Study the drawing (mm; zero at the part's minimum x, y, z) and answer. Coordinates: 2 decimals unless noted, no trailing zeros. Loops run counter-clockwise (first coordinate to the right, second up) from the corner with the lowest first, then second, coordinate; pieces in that order, holes last. Notation, with made-up numbers: M 28.25,76 L 49.25,76 A24 ccw 49.25,106 Z; hole C 52,31.25 d1. An arc over 180 degrees is marked long. Use one line per item in the form item = value. Start each with the question number.
1. The part is cut by section C-C (y = 147.5). Give the vertices of the cut face in (x, z).
2. Find the intervals of material crossed by probe 1 along Z at (x, y) = (9.5, 131); probe 2 along Z at (x, y) = (2.5, 76), in increasing order. Write a range as [from, to].
3. Flat-ended cylindrical pins translate along their axes: pin 1 (5 mm diameter, centred on y = 78.5, z = 21.5, fed in from -X); pin 2 (5 mm diameter, centred on x = 7, y = 114.5, fed in from -Z). Find the tip coordinate at first contact, or state that the pin passes through.
4. The part is cut by section B-B (x = 7.75). Give the vertices of the cut face in (y, z), plus the area to 3 significant figures.
5. The part is cut by section A-A (z = 14.5). Give the vertices of the cut face in (x, y).
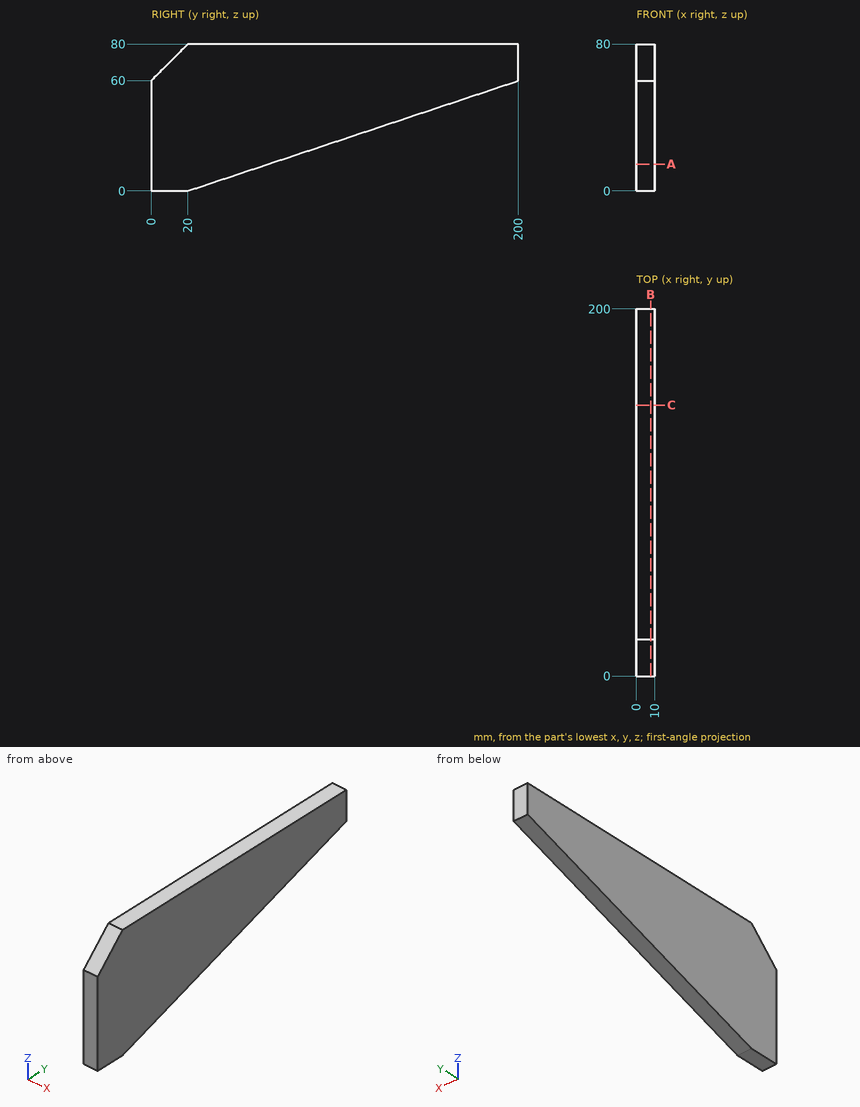
Computed values:
q1.outline = M 0,42.5 L 10,42.5 L 10,80 L 0,80 Z
q2.probe_1 = [37, 80]
q2.probe_2 = [18.67, 80]
q3.pin_1 = 0
q3.pin_2 = 30.67
q4.outline = M 0,0 L 20,0 L 200,60 L 200,80 L 20,80 L 0,60 Z
q4.area = 10,400 mm²
q5.outline = M 0,0 L 10,0 L 10,63.5 L 0,63.5 Z
